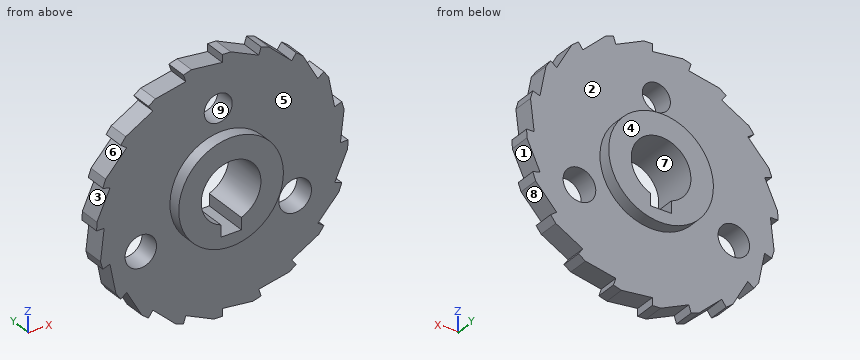
from build123d import *

# Parameters (mm, degrees)
RATCHET_WHEEL_BODY_20T_DEPTH = 10
HUB_BOSS_50_DEPTH            = 6
HUB_BOSS_50_DEPTH_BACK       = 16
HUB_SKETCH_R                 = 25
KEYED_SHAFT_BORE_DEPTH       = 57
THROUGH_HOLES_3X_DEPTH       = 57
THROUGH_HOLES_3X_DEPTH_BACK  = 57
THROUGH_HOLES_SKETCH_R       = 7.52194346
THROUGH_HOLES_SKETCH_R_2     = 7.800691594
THROUGH_HOLES_SKETCH_R_3     = 6.694831741


with BuildPart() as part:
    # Ratchet Tooth Profile Sketch → Ratchet Wheel Body 20T (new body)
    with BuildSketch(Plane(origin=(0, 0, 0), x_dir=(1, 0, 0), z_dir=(0, 1, 0))):
        Polygon((-14.697659706, -58.171976064), (0, -56.403789421), (0, -60), (3.997824162, -59.866663528), (17.429729478, -53.643191472), (18.541019662, -57.063390978), (22.301973147, -55.701184851), (23.837157922, -54.276602012), (33.153315595, -45.631624189), (35.267115138, -48.541019662), (38.423049613, -46.083286107), (45.631624189, -33.153315595), (48.541019662, -35.267115138), (50.783010274, -31.954434238), (53.643191472, -17.429729478), (57.063390978, -18.541019662), (58.171976064, -14.697659706), (56.403789421, 0), (60, 0), (59.866663528, 3.997824162), (53.643191472, 17.429729478), (57.063390978, 18.541019662), (55.701184851, 22.301973147), (45.631624189, 33.153315595), (48.541019662, 35.267115138), (46.083286107, 38.423049613), (33.153315595, 45.631624189), (35.267115138, 48.541019662), (31.954434238, 50.783010274), (17.429729478, 53.643191472), (18.541019662, 57.063390978), (14.697659706, 58.171976064), (0, 56.403789421), (0, 60), (-3.997824162, 59.866663528), (-17.429729478, 53.643191472), (-18.541019662, 57.063390978), (-22.301973147, 55.701184851), (-33.153315595, 45.631624189), (-35.267115138, 48.541019662), (-38.423049613, 46.083286107), (-45.631624189, 33.153315595), (-48.541019662, 35.267115138), (-50.783010274, 31.954434238), (-53.643191472, 17.429729478), (-57.063390978, 18.541019662), (-58.171976064, 14.697659706), (-56.403789421, 0), (-60, 0), (-59.866663528, -3.997824162), (-53.643191472, -17.429729478), (-57.063390978, -18.541019662), (-55.701184851, -22.301973147), (-45.631624189, -33.153315595), (-48.541019662, -35.267115138), (-46.083286107, -38.423049613), (-33.153315595, -45.631624189), (-35.267115138, -48.541019662), (-31.954434238, -50.783010274), (-17.429729478, -53.643191472), (-18.541019662, -57.063390978), align=None)
    extrude(amount=RATCHET_WHEEL_BODY_20T_DEPTH)

    # Hub Sketch → Hub Boss Ø50 (add, two sides: drawn at the far end of the back side and taken through both)
    with BuildSketch(Plane(origin=(0, 10, 0), x_dir=(1, 0, 0), z_dir=(0, 1, 0)).offset(-HUB_BOSS_50_DEPTH_BACK)):
        with Locations(Location((0, 0, 0), (0, 0, 270))):
            Circle(HUB_SKETCH_R)
    extrude(amount=HUB_BOSS_50_DEPTH + HUB_BOSS_50_DEPTH_BACK)

    # Keyed Bore Sketch → Keyed Shaft Bore (cut)
    with BuildSketch(Plane(origin=(0, 16, 0), x_dir=(1, 0, 0), z_dir=(0, 1, 0))):
        with BuildLine():
            Line((4.898606828, 13.381560116), (4.937062937, 13.381560116))
            Line((4.937062937, 13.381560116), (4.937062937, 19.059359245))
            Line((4.937062937, 19.059359245), (-4.898606828, 19.059359245))
            Line((-4.898606828, 19.059359245), (-4.898606828, 13.381560116))
            ThreePointArc((-4.898606828, 13.381560116), (0, -14.25), (4.898606828, 13.381560116))
        make_face()
    extrude(amount=-KEYED_SHAFT_BORE_DEPTH, mode=Mode.SUBTRACT)

    # Through Holes Sketch → Through Holes 3x (cut, two sides: drawn at the far end of the back side and taken through both)
    with BuildSketch(Plane(origin=(0, 0, 0), x_dir=(1, 0, 0), z_dir=(0, 1, 0)).offset(-THROUGH_HOLES_3X_DEPTH_BACK)):
        with Locations(Location((-38.922426411, 16.763050903, 0), (0, 0, 270))):
            Circle(THROUGH_HOLES_SKETCH_R)
        with Locations(Location((34.789071394, 16.763050903, 0), (0, 0, 270))):
            Circle(THROUGH_HOLES_SKETCH_R_2)
        with Locations(Location((-1.951862091, -36.052040982, 0), (0, 0, 270))):
            Circle(THROUGH_HOLES_SKETCH_R_3)
    extrude(amount=THROUGH_HOLES_3X_DEPTH + THROUGH_HOLES_3X_DEPTH_BACK, mode=Mode.SUBTRACT)


solid = part.part
CAD build for the part. Positions are in the model's coordinates, mm. Face numbers are marked on the shaded views. A direction names the side the tool comes from. Round coordinates to 2 decimals unless told otherwise and drop trailing zeros. Loops run counter-clockwise (first coordinate to the right, second up) from the corner with the lowest first, then second, coordinate; pieces in that order, holes last.
(1) Which spindle directions (+Z, -Z, +X, -X, +Y, -Y) get a long thin tool onto all of the face, cutting with end or side? Do the marked faces 1, 2, 3, 4 and 5. Say none if no direction does.
(2) Drop flat-ended pins along their axis: pin 1 (3 mm diameter, centred on x = -1, y = 6, fed in from +Z); pin 2 (12 mm diameter, centred on x = 35.5, z = -28.5, fed in from +Y); pin 3 (8 mm diameter, centred on y = 6, z = -8.5, fed in from -X); pin 4 (6 mm diameter, centred on x = -22, y = 5.5, fed in from -Z). Give the stop position or say it passes through.
(3) Two-plate mould, pull along X, no slides. Class the marked faces 6, 7, 8 and 9: +X half, -X half, draft (parallel to the pull), parting line (faces both ways), or undercut.
(4) Cut at D-D (y = 5). State how many separate pieces and enclosed holes the cut face has, plus the area to 3 significant figures.
(5) Cut at C-C (z = -7). Give the cut face in (x, y).
(6) Wall check: line 1 along Y through (x, z) = (22.5, -32.5); line 2 along Z through (x, y) = (35, 8.5); line 3 along X through (y, z) = (1.25, 42). Give the ranges that are in metal, low to high.
(7) Cut at A-A (z = 9). Give the cut face in (x, y).
Findings below:
1. face 1: +X, +Y, -Y
1. face 2: +Y
1. face 3: -X, +Y, -Y
1. face 4: +Z, -Z, +X, -X, +Y
1. face 5: -Y
2. pin 1: stops at z = 60
2. pin 2: stops at y = 10
2. pin 3: stops at x = -57.91
2. pin 4: stops at z = -56.9
3. face 6: -X half
3. face 7: undercut
3. face 8: +X half
3. face 9: undercut
4. separate pieces: 1
4. enclosed holes: 4
4. area: 9,490 mm2
5. outline: (-57.25, 0) - (-24, 0) - (-24, -6) - (-12.41, -6) - (-12.41, 16) - (-24, 16) - (-24, 10) - (-57.25, 10) - close; (12.41, -6) - (24, -6) - (24, 0) - (58.48, 0) - (58.48, 10) - (24, 10) - (24, 16) - (12.41, 16) - close
6. line 1: y = 0 to 10
6. line 2: z = -48.72 to -48.17, -44.6 to -24.56, -8.97 to 48.17
6. line 3: x = -39.67 to -5.02, 1.12 to 40.7
7. outline: (-57.55, 0) - (-23.32, 0) - (-23.32, -6) - (-11.05, -6) - (-11.05, 16) - (-23.32, 16) - (-23.32, 10) - (-57.55, 10) - close; (11.05, -6) - (23.32, -6) - (23.32, 0) - (57.49, 0) - (57.49, 10) - (23.32, 10) - (23.32, 16) - (11.05, 16) - close
